Design review of the part built by this model. Coordinates are the model's own, in mm. Round coordinates to 2 decimals unless told otherwise and drop trailing zeros. Loops run counter-clockwise (first coordinate to the right, second up) from the corner with the lowest first, then second, coordinate; pieces in that order, holes last. Notation, with made-up numbers: (48, 26) -> (78, 26) arc R37 ccw to (78, 63) -> close; hole circle Ø1 at (-1.75, -21.5). An arc over 180 degrees is marked (long way). Answer as CSV lines item,"result". Start each with the question number.
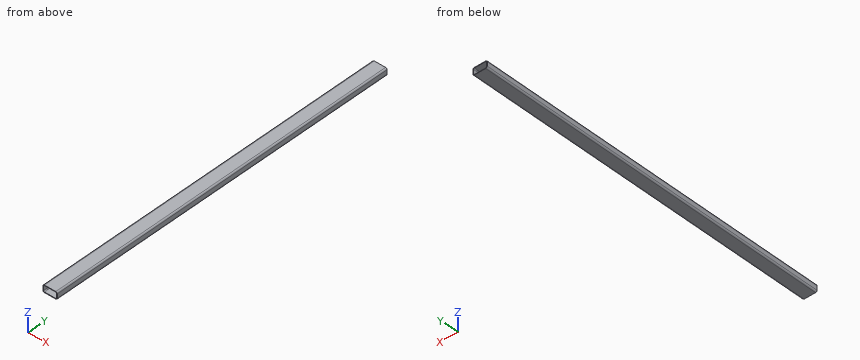
```python
from build123d import *

# Parameters (mm, degrees)
EXTRUDE_THIN1_DEPTH = 1265


with BuildPart() as part:
    # Sketch1 → Extrude-Thin1 (new, symmetric)
    with BuildSketch(Plane(origin=(0, 0, 0), x_dir=(1, 0, 0), z_dir=(0, 1, 0))):
        with BuildLine():
            Line((-40, 25), (40, 25))
            ThreePointArc((40, 25), (47.071067812, 22.071067812), (50, 15))
            Line((50, 15), (50, -15))
            ThreePointArc((50, -15), (47.071067812, -22.071067812), (40, -25))
            Line((40, -25), (-40, -25))
            ThreePointArc((-40, -25), (-47.071067812, -22.071067812), (-50, -15))
            Line((-50, -15), (-50, 15))
            ThreePointArc((-50, 15), (-47.071067812, 22.071067812), (-40, 25))
        make_face()
        with BuildLine():
            Line((-40, 21), (40, 21))
            ThreePointArc((40, 21), (44.242640687, 19.242640687), (46, 15))
            Line((46, 15), (46, -15))
            ThreePointArc((46, -15), (44.242640687, -19.242640687), (40, -21))
            Line((40, -21), (-40, -21))
            ThreePointArc((-40, -21), (-44.242640687, -19.242640687), (-46, -15))
            Line((-46, -15), (-46, 15))
            ThreePointArc((-46, 15), (-44.242640687, 19.242640687), (-40, 21))
        make_face(mode=Mode.SUBTRACT)
    extrude(amount=EXTRUDE_THIN1_DEPTH, both=True)


solid = part.part
```
Q1. Add section A-A, the plane x = 19. Give the boundary of the cut face in (y, z), and give its area (3 significant figures).
Q2. To check wall thickness, follow probe 1 along Z at (x, y) = (6.5, 71.5); probe 2 along X at (y, z) = (-645, 10); probe 3 along X at (y, z) = (-569.5, 20.5). State the ranges of each line that lie inside material, in increasing order. Write a range as from..to.
Q3. Add section B-B, the plane y = -617.5. Give the boundary of the cut face in (x, z), and give its area (3 significant figures).
Q4. Add section C-C, the plane z = -4. Give the boundary of the cut face in (x, y).
Worked answers:
1,outline,"(-1265, -25) -> (1265, -25) -> (1265, -21) -> (-1265, -21) -> close; (-1265, 21) -> (1265, 21) -> (1265, 25) -> (-1265, 25) -> close"
1,area,"20,200 mm^2"
2,probe 1,"z = -25..-21, 21..25"
2,probe 2,"x = -50..-46, 46..50"
2,probe 3,"x = -48.35..-42.4, 42.4..48.35"
3,outline,"(-50, -15) arc R10 ccw to (-40, -25) -> (40, -25) arc R10 ccw to (50, -15) -> (50, 15) arc R10 ccw to (40, 25) -> (-40, 25) arc R10 ccw to (-50, 15) -> close; hole (-46, -15) arc R6 ccw to (-40, -21) -> (40, -21) arc R6 ccw to (46, -15) -> (46, 15) arc R6 ccw to (40, 21) -> (-40, 21) arc R6 ccw to (-46, 15) -> close"
3,area,"1,080 mm^2"
4,outline,"(-50, -1265) -> (-46, -1265) -> (-46, 1265) -> (-50, 1265) -> close; (46, -1265) -> (50, -1265) -> (50, 1265) -> (46, 1265) -> close"
